from build123d import *

# Parameters (mm, degrees)
SKETCH_1_R              = 15
EXTRUDE_1_DEPTH         = 40
HOLE_WIZARD_M10_1_D     = 8.5
HOLE_WIZARD_M10_1_DEPTH = 20
HOLE_WIZARD_M10_1_TIP   = 2.553657631
SKETCH_4_R              = 6
EXTRUDE_2_DEPTH         = 15


with BuildPart() as part:
    # 草图1 → 凸台-拉伸1 (new, symmetric)
    with BuildSketch(Plane.XY):
        Circle(SKETCH_1_R)
    extrude(amount=EXTRUDE_1_DEPTH, both=True)

    # M10 螺纹孔1
    with Locations(Plane(origin=(0, 0, -40), x_dir=(-1, 0, 0), z_dir=(0, 0, -1))):
        with Locations((0, 0)):
            Hole(HOLE_WIZARD_M10_1_D / 2, depth=HOLE_WIZARD_M10_1_DEPTH)
            with Locations((0, 0, -(HOLE_WIZARD_M10_1_DEPTH + HOLE_WIZARD_M10_1_TIP / 2))):  # 118° drill point
                Cone(0, HOLE_WIZARD_M10_1_D / 2, HOLE_WIZARD_M10_1_TIP, mode=Mode.SUBTRACT)

    # 草图4 → 凸台-拉伸2 (add)
    with BuildSketch(Plane.XY.offset(40)):
        Circle(SKETCH_4_R)
    extrude(amount=EXTRUDE_2_DEPTH)


solid = part.part
Source: CAD feature listing. Evaluate the final solid. Frame: model axes, mm. A direction names the side the tool comes from. Round coordinates to 2 decimals unless told otherwise and drop trailing zeros. Loops run counter-clockwise (first coordinate to the right, second up) from the corner with the lowest first, then second, coordinate; pieces in that order, holes last. Notation, with made-up numbers: (26.5, 54.25) - (63.5, 54.25) arc R13 ccw to (63.5, 73.25) - close; hole circle Ø11 at (-26.5, -16). An arc over 180 degrees is marked (long way). Write item = value, one per line. Start each with the question number.
Item 1: First-contact query: pin 1 Ø5 at (y, z) = (-4, 3.5) entering from -X; pin 2 Ø10 at (y, z) = (12, -13.5) entering from +X; pin 3 Ø1.5 at (y, z) = (8.5, 1.5) entering from -X. Flat tips, straight axial feed; report the tip coordinate or a pass-through.
Item 2: Section query C-C on x = -11.25. Output: boundary loops of the cut face in (y, z), plus the area to 3 significant figures.
Item 3: Reachability of faces 4 (the face through (6.5, 0.2, 40)), 5 (the face through (0.16, -0.72, -17.89)) from +Z, -Z, +X, -X, +Y, -Y: full face, straight path, thin tool, end or side. Return the list, or none.
Item 4: Section query A-A on z = 35. Output: boundary loops of the cut face in (x, y), plus the area to 3 significant figures.
Item 5: Section query B-B on y = -12. Output: boundary loops of the cut face in (x, z).
Item 6: Material intervals for line 1 (Y direction, x = 0, z = -30.5); line 2 (Z direction, x = -7, y = -4.5); line 3 (Y direction, x = 6.5, z = 7), sorted ascending.
Item 7: Mould query, pull axis Y, two halves, no side actions, for faces 1 (the face through (2.285, 3.584, -29.86)), 2 (the face through (3.12, -3.12, -40)), 3 (the face through (-6, 0, 47)). Classes: released by +Y, released by -Y, zero draft, split by the parting line, or undercut.
Results list:
q1.pin_1 = -14.92
q1.pin_2 = 13.27
q1.pin_3 = -12.84
q2.outline = (-9.92, -40) - (9.92, -40) - (9.92, 40) - (-9.92, 40) - close
q2.area = 1,590 mm²
q3.face_4 = +Z
q3.face_5 = -Z
q4.outline = circle Ø30 at (0, 0)
q4.area = 707 mm²
q5.outline = (-9, -40) - (9, -40) - (9, 40) - (-9, 40) - close
q6.line_1 = -15 to -4.25, 4.25 to 15
q6.line_2 = -40 to 40
q6.line_3 = -13.52 to 13.52
q7.face_1 = undercut
q7.face_2 = zero draft
q7.face_3 = split by the parting line
